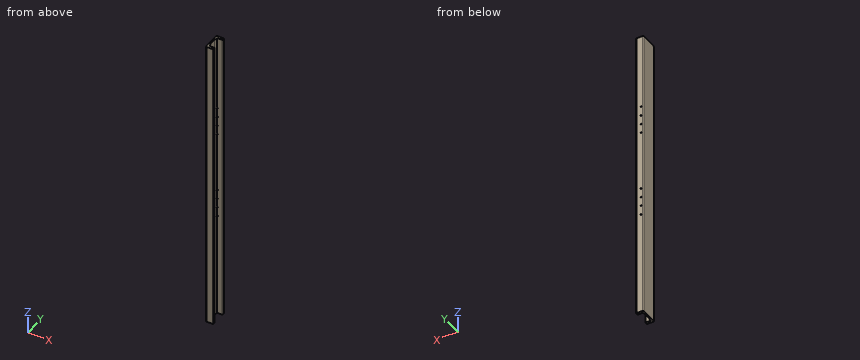
from build123d import *

# Parameters (mm, degrees)
BOSS_EXTRUDE1_DEPTH   = 1430
M6_TAPPED_HOLE1_D     = 5
M6_TAPPED_HOLE1_DEPTH = 15
M6_TAPPED_HOLE1_TIP   = 1.502151548


with BuildPart() as part:
    # Sketch1 → Boss-Extrude1 (new body)
    with BuildSketch(Plane.XY):
        with BuildLine():
            Line((-3, 0), (-32, 0))
            ThreePointArc((-32, 0), (-34.828427125, -1.171572875), (-36, -4))
            Line((-36, -4), (-36, -82.5))
            ThreePointArc((-36, -82.5), (-34.828427125, -85.328427125), (-32, -86.5))
            Line((-32, -86.5), (-3, -86.5))
            ThreePointArc((-3, -86.5), (-0.878679656, -85.621320344), (0, -83.5))
            Line((0, -83.5), (0, -77))
            ThreePointArc((0, -77), (-0.732233047, -75.232233047), (-2.5, -74.5))
            Line((-2.5, -74.5), (-26, -74.5))
            Line((-26, -74.5), (-29, -59.5))
            Line((-29, -59.5), (-29, -27))
            Line((-29, -27), (-26, -12))
            Line((-26, -12), (-2.5, -12))
            ThreePointArc((-2.5, -12), (-0.732233047, -11.267766953), (0, -9.5))
            Line((0, -9.5), (0, -3))
            ThreePointArc((0, -3), (-0.878679656, -0.878679656), (-3, 0))
        make_face()
    extrude(amount=BOSS_EXTRUDE1_DEPTH)

    # M6 Tapped Hole1
    with Locations(Plane(origin=(0, 0, 0), x_dir=(1, 0, 0), z_dir=(0, 1, 0))):
        with Locations((-25, -505), (-25, -550), (-25, -595), (-25, -640), (-25, -930), (-25, -975), (-25, -1020), (-25, -1065)):
            Hole(M6_TAPPED_HOLE1_D / 2, depth=M6_TAPPED_HOLE1_DEPTH)
            with Locations((0, 0, -(M6_TAPPED_HOLE1_DEPTH + M6_TAPPED_HOLE1_TIP / 2))):  # 118° drill point
                Cone(0, M6_TAPPED_HOLE1_D / 2, M6_TAPPED_HOLE1_TIP, mode=Mode.SUBTRACT)


solid = part.part
For this review, take the finished solid that the model builds, in its own axes (mm). Coordinates: 2 decimals unless noted, no trailing zeros. Order: outer loops, then holes, each group sorted by start corner. A loop starts at its lowest first (then second) coordinate and runs counter-clockwise, first axis right, second up. Notation, with made-up numbers: (-17, 72) -> (17, 72) arc R16 cw to (17, 83) -> close; hole circle Ø11 at (-34, 9). An arc over 180 degrees is marked (long way). Return JSON: item names as keys, results as strings.
1. We need section B-B on z = 224. Write out the cut boundary in (x, y), and give its area (3 significant figures).
Answer block:
{"outline": "(-36, -82.5) arc R4 ccw to (-32, -86.5) -> (-3, -86.5) arc R3 ccw to (0, -83.5) -> (0, -77) arc R2.5 ccw to (-2.5, -74.5) -> (-26, -74.5) -> (-29, -59.5) -> (-29, -27) -> (-26, -12) -> (-2.5, -12) arc R2.5 ccw to (0, -9.5) -> (0, -3) arc R3 ccw to (-3, 0) -> (-32, 0) arc R4 ccw to (-36, -4) -> close", "area": "1,330 mm²"}
2. For pin 1 Ø4.5 at (x, z) = (-25, 595) entering from +Y; pin 2 Ø16 at (y, z) = (-49.5, 933.5) entering from +X, all flat-tipped, find the tip position at first contact; note any pin that passes through.
Answer block:
{"pin 1": "y = -15.15", "pin 2": "x = -29"}
3. We need section A-A on x = -15.5. Write out the cut boundary in (y, z).
Answer block:
{"outline": "(-86.5, 0) -> (-74.5, 0) -> (-74.5, 1430) -> (-86.5, 1430) -> close; (-12, 0) -> (0, 0) -> (0, 1430) -> (-12, 1430) -> close"}
4. We need section C-C on y = -42.5. Write out the cut boundary in (x, z), and give its area (3 significant figures).
Answer block:
{"outline": "(-36, 0) -> (-29, 0) -> (-29, 1430) -> (-36, 1430) -> close", "area": "10,000 mm²"}
5. For line 1 (Y direction, x = -11.5, z = 1048.5); line 2 (X direction, y = -53, z = 1206.5); line 3 (X direction, y = -3.75, z = 505), list the stretches that pass through material, from the lowest coordinate up. Write a range as from..to.
Answer block:
{"line 1": "-86.5..-74.5, -12..0", "line 2": "-36..-29", "line 3": "-35.99..-27.5, -22.5..0"}
